```python
from build123d import *

# Parameters (mm, degrees)
EXTRUDE1_DEPTH                                       = 100
HOLE_SIZE_PER_SOCKET_HEAD_CAP_SCREW_TYPE_D           = 5.5
HOLE_SIZE_PER_SOCKET_HEAD_CAP_SCREW_TYPE_CBORE_D     = 10
HOLE_SIZE_PER_SOCKET_HEAD_CAP_SCREW_TYPE_CBORE_DEPTH = 5.7


with BuildPart() as part:
    # Sketch1 → Extrude1 (new body)
    with BuildSketch(Plane.XY):
        with BuildLine():
            Line((0, 13.5), (0, 17))
            Line((0, 17), (1, 18))
            Line((1, 18), (19, 18))
            Line((19, 18), (20, 17))
            Line((20, 17), (20, 13.5))
            ThreePointArc((20, 13.5), (17.5, 11), (20, 8.5))
            Line((20, 8.5), (20, 1))
            Line((20, 1), (19, 0))
            Line((19, 0), (1, 0))
            Line((1, 0), (0, 1))
            Line((0, 1), (0, 8.5))
            ThreePointArc((0, 8.5), (2.5, 11), (0, 13.5))
        make_face()
    extrude(amount=EXTRUDE1_DEPTH)

    # Hole size per socket head cap screw type 1 (through all)
    with Locations(Plane(origin=(10, 18, 20), x_dir=(0, 0, 1), z_dir=(0, 1, 0))):
        with Locations((0, 0), (60, 0)):
            CounterBoreHole(HOLE_SIZE_PER_SOCKET_HEAD_CAP_SCREW_TYPE_D / 2, HOLE_SIZE_PER_SOCKET_HEAD_CAP_SCREW_TYPE_CBORE_D / 2, HOLE_SIZE_PER_SOCKET_HEAD_CAP_SCREW_TYPE_CBORE_DEPTH)


solid = part.part
```
Source: CAD feature listing. Evaluate the final solid. Frame: model axes, mm. A direction names the side the tool comes from. Round coordinates to 2 decimals unless told otherwise and drop trailing zeros. Order: outer loops, then holes, each group sorted by start corner. A loop starts at its lowest first (then second) coordinate and runs counter-clockwise, first axis right, second up. Notation, with made-up numbers: (-10.5, -9) -> (8.5, -9) arc R5 cw to (8.5, -1) -> close; hole circle Ø5 at (5.25, -17). An arc over 180 degrees is marked (long way). Use CSV: the item, a comma, the result in double quotes.
(1) Section A-A on x = 10. Return the cut outline in (y, z).
Report:
outline,"(0, 0) -> (18, 0) -> (18, 15) -> (12.3, 15) -> (12.3, 17.25) -> (0, 17.25) -> close; (0, 22.75) -> (12.3, 22.75) -> (12.3, 25) -> (18, 25) -> (18, 75) -> (12.3, 75) -> (12.3, 77.25) -> (0, 77.25) -> close; (0, 82.75) -> (12.3, 82.75) -> (12.3, 85) -> (18, 85) -> (18, 100) -> (0, 100) -> close"
(2) Access query for faces 1 (the face through (8.085, 15.19, 84.619)), 2 (the face through (2.5, 10.9, 49.3)). Directions: +Z, -Z, +X, -X, +Y, -Y. A direction counts if a zero-diameter tool reaches every point of the face in a straight line with its end or side. Return the directions, or none.
Report:
face 1,"+Y"
face 2,"+Z, -Z, -X"
(3) Ray query, L1, parallel to Z at x = 9.75, y = 1.75; L2, parallel to X at y = 14.3, z = 80; L3, parallel to X at y = 2.5, z = 80. Return the intervals inside material, ascending.
Report:
L1,"0 to 17.26, 22.74 to 77.26, 82.74 to 100"
L2,"0 to 5, 15 to 20"
L3,"0 to 7.25, 12.75 to 20"
(4) Pull-direction query (Z, two-part tool) for faces 3 (the face through (10.121, 6.064, 22.747)), 4 (the face through (10, 9, 0)), 5 (the face through (17.5, 11.1, 49.3)); classes: +Z half, -Z half, draft (parallel to the pull), parting line (faces both ways), or undercut.
Report:
face 3,"undercut"
face 4,"-Z half"
face 5,"draft"
(5) Section C-C on y = 11. Return the cut outline in (x, z), and give its area (3 significant figures).
Report:
outline,"(2.5, 0) -> (17.5, 0) -> (17.5, 100) -> (2.5, 100) -> close; hole circle Ø5.5 at (10, 20); hole circle Ø5.5 at (10, 80)"
area,"1,450 mm^2"
(6) First-contact query: pin 1 Ø6 at (x, z) = (10, 80) entering from +Y; pin 2 Ø2 at (x, z) = (7, 51) entering from -Y. Flat tips, straight axial feed; report the tip coordinate or a pass-through.
Report:
pin 1,"y = 12.3"
pin 2,"y = 0"
(7) Section B-B on z = 80. Return the cut outline in (x, y).
Report:
outline,"(0, 1) -> (1, 0) -> (7.25, 0) -> (7.25, 12.3) -> (5, 12.3) -> (5, 18) -> (1, 18) -> (0, 17) -> (0, 13.5) arc R2.5 cw to (0, 8.5) -> close; (12.75, 0) -> (19, 0) -> (20, 1) -> (20, 8.5) arc R2.5 cw to (20, 13.5) -> (20, 17) -> (19, 18) -> (15, 18) -> (15, 12.3) -> (12.75, 12.3) -> close"
(8) Section D-D on z = 30. Return the cut outline in (x, y).
Report:
outline,"(0, 1) -> (1, 0) -> (19, 0) -> (20, 1) -> (20, 8.5) arc R2.5 cw to (20, 13.5) -> (20, 17) -> (19, 18) -> (1, 18) -> (0, 17) -> (0, 13.5) arc R2.5 cw to (0, 8.5) -> close"
